```python
from build123d import *

# Parameters (mm, degrees)
SKETCH1_W             = 161
SKETCH1_H             = 120
BOSS_EXTRUDE1_DEPTH   = 30
CUT_EXTRUDE1_DEPTH    = 105.786688086
M16_TAPPED_HOLE1_D    = 14
M8_TAPPED_HOLE1_D     = 6.8
M8_TAPPED_HOLE1_DEPTH = 19.75
M8_TAPPED_HOLE1_TIP   = 2.042926105
SKETCH7_R             = 4
CUT_EXTRUDE2_DEPTH    = 15
CHAMFER1_SIZE         = 15
CHAMFER2_SIZE         = 5


with BuildPart() as part:
    # Sketch1 → Boss-Extrude1 (new body)
    with BuildSketch(Plane(origin=(0, 0, 0), x_dir=(1, 0, 0), z_dir=(0, 1, 0))):
        Rectangle(SKETCH1_W, SKETCH1_H)
    extrude(amount=BOSS_EXTRUDE1_DEPTH)

    # Sketch2 → Cut-Extrude1 (cut, through all)
    with BuildSketch(Plane(origin=(0, 30, 0), x_dir=(1, 0, 0), z_dir=(0, 1, 0))):
        with BuildLine():
            Line((-22, 10), (-22, 60))
            Line((-22, 60), (22, 60))
            Line((22, 60), (22, 10))
            ThreePointArc((22, 10), (0, -12), (-22, 10))
        make_face()
    extrude(amount=-CUT_EXTRUDE1_DEPTH, mode=Mode.SUBTRACT)

    # M16 Tapped Hole1 (through all)
    with Locations(Plane(origin=(0, 30, 0), x_dir=(-1, 0, 0), z_dir=(0, 1, 0))):
        with Locations((65, -15), (-65, -15)):
            Hole(M16_TAPPED_HOLE1_D / 2)

    # M8 Tapped Hole1
    with Locations(Plane.XY.offset(60)):
        with Locations((70.5, 15), (-70.5, 15)):
            Hole(M8_TAPPED_HOLE1_D / 2, depth=M8_TAPPED_HOLE1_DEPTH)
            with Locations((0, 0, -(M8_TAPPED_HOLE1_DEPTH + M8_TAPPED_HOLE1_TIP / 2))):  # 118° drill point
                Cone(0, M8_TAPPED_HOLE1_D / 2, M8_TAPPED_HOLE1_TIP, mode=Mode.SUBTRACT)

    # Sketch7 → Cut-Extrude2 (cut)
    with BuildSketch(Plane.XY.offset(60)):
        with Locations((-35, 15)):
            Circle(SKETCH7_R)
        with Locations((35, 15)):
            Circle(SKETCH7_R)
    extrude(amount=-CUT_EXTRUDE2_DEPTH, mode=Mode.SUBTRACT)

    # Chamfer1
    chamfer1_edges = [part.edges().sort_by_distance(p)[0] for p in [
        (-80.5, 15, -60),
        (80.5, 15, -60),
    ]]
    chamfer(chamfer1_edges, length=CHAMFER1_SIZE)

    # Chamfer2
    chamfer2_edges = [part.edges().sort_by_distance(p)[0] for p in [
        (-22, 15, -60),
        (22, 15, -60),
    ]]
    chamfer(chamfer2_edges, length=CHAMFER2_SIZE)


solid = part.part
```
Build history of the part. All positions in model axes, mm. A direction names the side the tool comes from. Give positions to 0.01 mm unless a question says otherwise; leave off trailing zeros. Loops run counter-clockwise (first coordinate to the right, second up) from the corner with the lowest first, then second, coordinate; pieces in that order, holes last.
Item 1: Pull direction Y, two halves, no side cores. Call faces 1 (the face through (71.06, 15.18, 38.56)), 2 (the face through (72.9, 14.8, -52.6)), 3 (the face through (-1.1, 0, 12.5)): released by +Y, released by -Y, zero draft, split by the parting line, or undercut.
Answers follow:
face 1: undercut
face 2: zero draft
face 3: released by -Y
Item 2: Slice it at A-A, the plane z = -15. List the corners of the cut face in (x, y).
Answers follow:
outline: (-80.5, 0) - (-72, 0) - (-72, 30) - (-80.5, 30) - close; (-58, 0) - (-22, 0) - (-22, 30) - (-58, 30) - close; (22, 0) - (58, 0) - (58, 30) - (22, 30) - close; (72, 0) - (80.5, 0) - (80.5, 30) - (72, 30) - close
Item 3: Drill centre lines: line 1 (Y direction, x = 70, z = 53); line 2 (X direction, y = 2, z = -26.5); line 3 (Z direction, x = 65, y = 23). Where is each one in solid material? Low to high.
Answers follow:
line 1: y = 0 to 11.64, 18.36 to 30
line 2: x = -80.5 to -22, 22 to 80.5
line 3: z = -60 to -22, -8 to 60
Item 4: Flat gauge pins, fed straight in: pin 1 (2 mm diameter, centred on x = 19, y = 12.5, fed in from -Z); pin 2 (5 mm diameter, centred on x = 35, y = 15, fed in from +Z); pin 3 (8 mm diameter, centred on x = 70.5, y = 15, fed in from +Z); pin 4 (5.5 mm diameter, centred on x = -70.5, y = 15, fed in from -Z). Where does each tip first touch, or does it go through?
Answers follow:
pin 1: stops at z = -0.83
pin 2: stops at z = 45
pin 3: stops at z = 60
pin 4: stops at z = -57.75
Item 5: Slice it at B-B, the plane x = -61. List the corners of the cut face in (y, z).
Answers follow:
outline: (0, -60) - (30, -60) - (30, -20.74) - (0, -20.74) - close; (0, -9.26) - (30, -9.26) - (30, 60) - (0, 60) - close
Item 6: Slice it at D-D, the plane x = -35. List the corners of the cut face in (y, z).
Answers follow:
outline: (0, -60) - (30, -60) - (30, 60) - (19, 60) - (19, 45) - (11, 45) - (11, 60) - (0, 60) - close
Item 7: Slice it at C-C, the plane y = 27.5. List the corners of the cut face in (x, z), and give its area (3 significant figures).
Answers follow:
outline: (-80.5, -45) - (-65.5, -60) - (-27, -60) - (-22, -55) - (-22, -10) arc R22 cw to (22, -10) - (22, -55) - (27, -60) - (65.5, -60) - (80.5, -45) - (80.5, 60) - (-80.5, 60) - close; hole circle Ø14 at (-65, -15); hole circle Ø14 at (65, -15)
area: 15,800 mm2
Item 8: Which spindle directions (+Z, -Z, +X, -X, +Y, -Y) get a long thin tool onto all of the face, cutting with end or side? Do faces 4 (the face through (32.05, 17.7, 52.6)), 5 (the face through (-1, 15, 60)), 6 (the face through (24, 15, -57)). Say none if no direction does.
Answers follow:
face 4: +Z
face 5: +Z, +X, -X, +Y, -Y
face 6: -Z, +Y, -Y
